CAD build for the part. Positions are in the model's coordinates, mm. Coordinates: 2 decimals unless noted, no trailing zeros. Write each loop counter-clockwise with the first axis right and the second up, starting at its lowest first coordinate (ties: lowest second). Pieces come first, ordered by that corner, then holes.
```python
from build123d import *

# Parameters (mm, degrees)
SKETCH_1_W            = 30
SKETCH_1_H            = 30
SKETCH_1_R            = 1.25
EXTRUDE_1_DEPTH       = 5
HOLE_WIZARD_7_0_7_1_D = 7


with BuildPart() as part:
    # 草图1 → 凸台-拉伸1 (new body)
    with BuildSketch(Plane.XY.offset(5)):
        Rectangle(SKETCH_1_W, SKETCH_1_H)
        with Locations(Location((-10, 10, 0), (0, 0, 180))):
            Circle(SKETCH_1_R, mode=Mode.SUBTRACT)
        with Locations(Location((10, 10, 0), (0, 0, 180))):
            Circle(SKETCH_1_R, mode=Mode.SUBTRACT)
    extrude(amount=-EXTRUDE_1_DEPTH)

    # Ø7.0 (7) 直径孔1 (through all)
    with Locations(Plane.XY.offset(5)):
        with Locations((10, 0), (-10, 0)):
            Hole(HOLE_WIZARD_7_0_7_1_D / 2)


solid = part.part
```
Item 1: Two-plate mould, pull along Y, no slides. Class faces 1 (the cylindrical face through (11.25, 9.95, 2.54)), 2 (the flat face through (15, 0, 3)), 3 (the cylindrical face through (-8.75, 9.95, 2.54)), 4 (the flat face through (0, -15, 3)): +Y half, -Y half, draft (parallel to the pull), parting line (faces both ways), or undercut.
Item 2: Saw through at A-A, the plane x = 10. Write the cut outline in (y, z), and give its area (4 significant figures).
Item 3: Saw through at B-B, the plane y = 10. Write the cut outline in (x, z), and give its area (3 significant figures).
Item 4: Saw through at C-C, the plane z = 2.05. Write the cut outline in (x, y), and give its area (3 significant figures).
Item 5: Flat gauge pin, fed straight in: pin 1 Ø2 at (x, y) = (-10, 10) entering from -Z. Where does the tip first touch, or does it go through?
Item 6: Wall check: line 1 along X through (y, z) = (10, 2.5); line 2 along Y through (x, z) = (10, 1.8); line 3 along X through (y, z) = (10.5, 2.55). Give the ranges that are in metal, low to high.
Working result:
1. face 1: undercut
1. face 2: draft
1. face 3: undercut
1. face 4: -Y half
2. outline: (-15, 0) - (-3.5, 0) - (-3.5, 5) - (-15, 5) - close; (3.5, 0) - (8.75, 0) - (8.75, 5) - (3.5, 5) - close; (11.25, 0) - (15, 0) - (15, 5) - (11.25, 5) - close
2. area: 102.5 mm2
3. outline: (-15, 0) - (-11.25, 0) - (-11.25, 5) - (-15, 5) - close; (-8.75, 0) - (8.75, 0) - (8.75, 5) - (-8.75, 5) - close; (11.25, 0) - (15, 0) - (15, 5) - (11.25, 5) - close
3. area: 125 mm2
4. outline: (-15, -15) - (15, -15) - (15, 15) - (-15, 15) - close; hole circle Ø7 at (-10, 0); hole circle Ø2.5 at (-10, 10); hole circle Ø7 at (10, 0); hole circle Ø2.5 at (10, 10)
4. area: 813 mm2
5. pin 1: passes through
6. line 1: x = -15 to -11.25, -8.75 to 8.75, 11.25 to 15
6. line 2: y = -15 to -3.5, 3.5 to 8.75, 11.25 to 15
6. line 3: x = -15 to -11.15, -8.85 to 8.85, 11.15 to 15
